Design review of the part shown in the three views and the two pictorial views. Dimensions are in mm from the part's minimum x, y and z. Coordinates: 2 decimals unless noted, no trailing zeros. Write each loop counter-clockwise with the first axis right and the second up, starting at its lowest first coordinate (ties: lowest second). Pieces come first, ordered by that corner, then holes. Notation, with made-up numbers: M -33.75,62.5 L 12.25,62.5 A26 ccw 12.25,84.5 Z; hole C 44.5,-11 d4. An arc over 180 degrees is marked long. Answer as a JSON object with one key per item and string values.
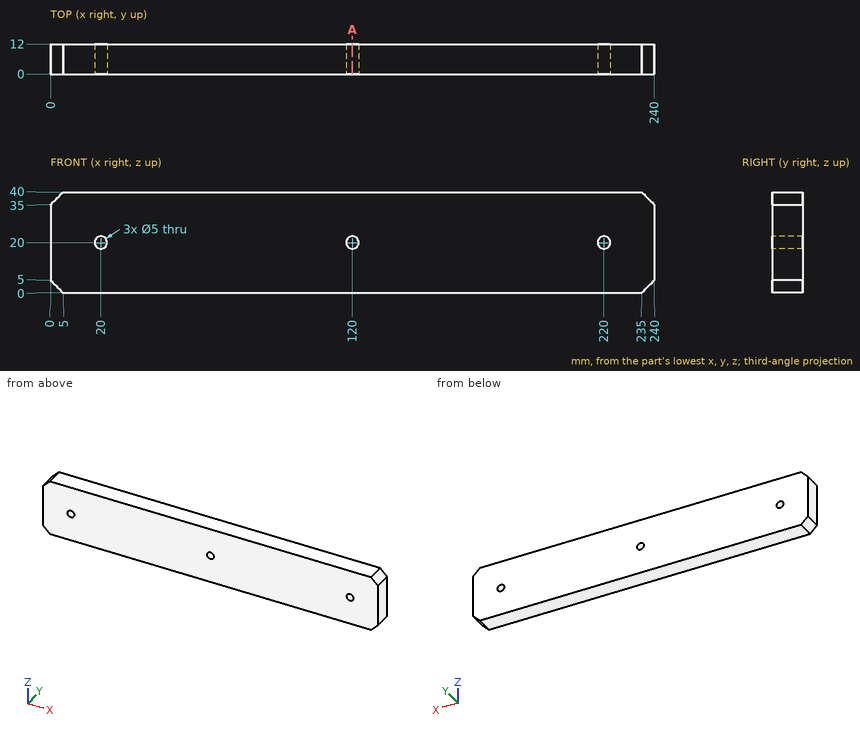
(1) Add section A-A on x = 120. Give the boundary of the cut face in (y, z).
Results list:
{"outline": "M 0,0 L 12,0 L 12,17.5 L 0,17.5 Z; M 0,22.5 L 12,22.5 L 12,40 L 0,40 Z"}
(2) Wall thickness on line 1 along Z through (x, y) = (220, 8.25); line 2 along Z through (x, y) = (222, 2); line 3 along X through (y, z) = (1, 2.5): over which ranges is each line inside the solid? List them lowest first. Write a range as from..to.
Results list:
{"line 1": "0..17.5, 22.5..40", "line 2": "0..18.5, 21.5..40", "line 3": "2.5..237.5"}
(3) For pin 1 Ø4 at (x, z) = (120, 20) entering from -Y, flat-tipped, find the tip position at first contact; note if it passes through.
Results list:
{"pin 1": "through"}
